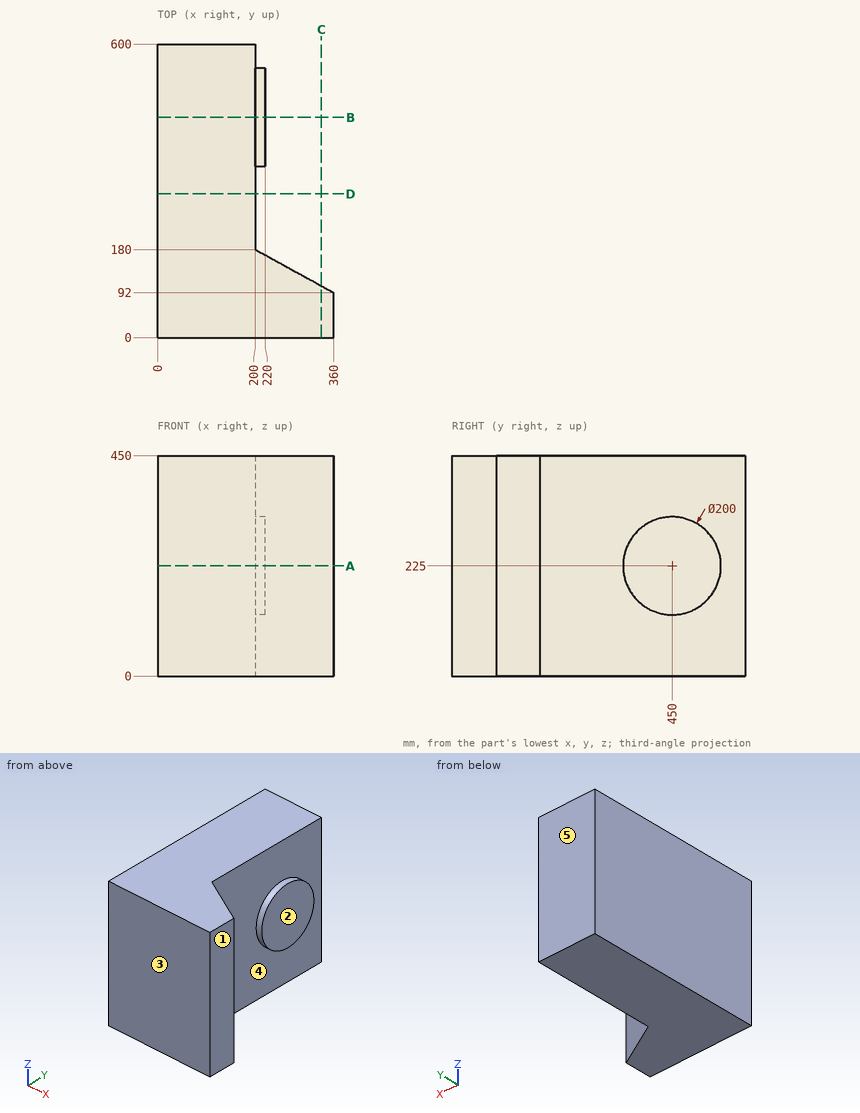
Part print with two shaded views. Sizes in mm from the minimum x, y, z corner. A direction names the side the tool comes from. Round coordinates to 2 decimals unless told otherwise and drop trailing zeros. Order: outer loops, then holes, each group sorted by start corner. A loop starts at its lowest first (then second) coordinate and runs counter-clockwise, first axis right, second up. Notation, with made-up numbers: M 8.25,58 L 33.25,58 A24 ccw 33.25,75 Z; hole C 16.25,75 d8. An arc over 180 degrees is marked long. Put each result on its own line as item: value. Start each with the question number.
1. Tool access for the marked faces 1 and 2: list every direction of +Z, -Z, +X, -X, +Y, -Y with a clear straight run to the whole face (end or side of a thin tool).
2. Drop flat-ended pins along their axis: pin 1 (5 mm diameter, centred on x = 223.5, z = 126, fed in from +Y); pin 2 (1.5 mm diameter, centred on y = 352.5, z = 225, fed in from +X). Give the stop position or say it passes through.
3. Slice it at B-B on y = 450. List the corners of the cut face in (x, z).
4. Slice it at D-D on y = 294. List the corners of the cut face in (x, z).
5. Slice it at A-A on z = 225. List the corners of the cut face in (x, y).
6. Slice it at C-C on x = 334.5. List the corners of the cut face in (y, z) (3 decimals).
7. Drill centre lines: probe 1 along X at (y, z) = (553, 268.5); probe 2 along Y at (x, z) = (207, 273); probe 3 along X at (y, z) = (533.5, 221). Where is each one in solid material? Low to high. Write a range as [from, to].
8. Two-plate mould, pull along Y, no slides. Class the marked faces 3, 4 and 5: +Y half, -Y half, draft (parallel to the pull), parting line (faces both ways), or undercut.
Findings:
1. face 1: +Z, -Z, +X, +Y, -Y
1. face 2: +Z, -Z, +X, +Y
2. pin 1: y = 168.45
2. pin 2: x = 220
3. outline: M 0,0 L 200,0 L 200,125 L 220,125 L 220,325 L 200,325 L 200,450 L 0,450 Z
4. outline: M 0,0 L 200,0 L 200,450 L 0,450 Z
5. outline: M 0,0 L 360,0 L 360,92 L 200,180 L 200,350 L 220,350 L 220,550 L 200,550 L 200,600 L 0,600 Z
6. outline: M 0,0 L 106.025,0 L 106.025,450 L 0,450 Z
7. probe 1: [0, 200]
7. probe 2: [0, 176.15], [362.27, 537.73]
7. probe 3: [0, 220]
8. face 3: -Y half
8. face 4: undercut
8. face 5: +Y half
